from build123d import *

# Parameters (mm, degrees)
SKETCH1_W             = 100
SKETCH1_H             = 100
BOSS_EXTRUDE1_DEPTH   = 10
SKETCH2_W             = 50
SKETCH2_H             = 10
CUT_EXTRUDE1_DEPTH    = 113.249721603
SKETCH3_W             = 50
SKETCH3_H             = 10
CUT_EXTRUDE2_DEPTH    = 113.249721603
FILLET1_R             = 10
SKETCH5_R             = 30
BOSS_EXTRUDE2_DEPTH   = 2
SKETCH6_W             = 50
SKETCH6_H             = 20
BOSS_EXTRUDE3_DEPTH   = 50
SKETCH7_W             = 50
SKETCH7_H             = 35
BOSS_EXTRUDE6_DEPTH   = 20
CHAMFER1_SIZE         = 2
M8_TAPPED_HOLE1_D     = 6.8
M8_TAPPED_HOLE1_DEPTH = 20.207073895
M8_TAPPED_HOLE1_TIP   = 2.042926105


with BuildPart() as part:
    # Sketch1 → Boss-Extrude1 (new body)
    with BuildSketch(Plane(origin=(0, 0, 0), x_dir=(1, 0, 0), z_dir=(0, 1, 0))):
        Rectangle(SKETCH1_W, SKETCH1_H)
    extrude(amount=BOSS_EXTRUDE1_DEPTH)

    # Sketch2 → Cut-Extrude1 (cut, through all)
    with BuildSketch(Plane.XY.offset(50)):
        Rectangle(SKETCH2_W, SKETCH2_H)
    extrude(amount=-CUT_EXTRUDE1_DEPTH, mode=Mode.SUBTRACT)

    # Sketch3 → Cut-Extrude2 (cut, through all)
    with BuildSketch(Plane(origin=(50, 0, 0), x_dir=(0, 0, -1), z_dir=(1, 0, 0))):
        Rectangle(SKETCH3_W, SKETCH3_H)
    extrude(amount=-CUT_EXTRUDE2_DEPTH, mode=Mode.SUBTRACT)

    # Fillet1
    fillet1_edges = [part.edges().sort_by_distance(p)[0] for p in [
        (50, 5, 50),
        (-50, 5, 50),
        (-50, 5, -50),
        (50, 5, -50),
    ]]
    fillet(fillet1_edges, radius=FILLET1_R)

    # Sketch4 → Revolve1 (revolve)
    with BuildSketch(Plane.XY):
        Polygon((0, 10), (0, 30), (30, 30), (40, 10), align=None)
    revolve(axis=Axis((0, 10, 0), (0, 1, 0)))

    # Sketch5 → Boss-Extrude2 (add)
    with BuildSketch(Plane(origin=(0, 30, 0), x_dir=(1, 0, 0), z_dir=(0, 1, 0))):
        with Locations(Location((0, 0, 0), (0, 0, 180))):
            Circle(SKETCH5_R)
    extrude(amount=BOSS_EXTRUDE2_DEPTH)

    # Sketch6 → Boss-Extrude3 (add)
    with BuildSketch(Plane(origin=(0, 0, 0), x_dir=(0, 0, -1), z_dir=(1, 0, 0))):
        with Locations((0, 20)):
            Rectangle(SKETCH6_W, SKETCH6_H)
    extrude(amount=BOSS_EXTRUDE3_DEPTH)

    # Sketch7 → Boss-Extrude6 (add)
    with BuildSketch(Plane(origin=(50, 0, 0), x_dir=(0, 0, -1), z_dir=(1, 0, 0))):
        with Locations((0, 22.5)):
            Rectangle(SKETCH7_W, SKETCH7_H)
    extrude(amount=BOSS_EXTRUDE6_DEPTH)

    # Chamfer1
    chamfer1_edges = [part.edges().sort_by_distance(p)[0] for p in [
        (70, 5, 0),
        (50, 40, 0),
        (60, 5, -25),
        (50, 35, -25),
        (60, 40, -25),
        (70, 22.5, -25),
        (70, 40, 0),
        (60, 5, 25),
        (70, 22.5, 25),
        (60, 40, 25),
        (50, 35, 25),
    ]]
    chamfer(chamfer1_edges, length=CHAMFER1_SIZE)

    # M8 Tapped Hole1
    with Locations(Plane(origin=(0, 10, 0), x_dir=(1, 0, 0), z_dir=(0, 1, 0))):
        with Locations((40, 40), (40, -40), (-40, -40), (-40, 40)):
            Hole(M8_TAPPED_HOLE1_D / 2, depth=M8_TAPPED_HOLE1_DEPTH)
            with Locations((0, 0, -(M8_TAPPED_HOLE1_DEPTH + M8_TAPPED_HOLE1_TIP / 2))):  # 118° drill point
                Cone(0, M8_TAPPED_HOLE1_D / 2, M8_TAPPED_HOLE1_TIP, mode=Mode.SUBTRACT)


solid = part.part
Verification items for the finished model (mm, model axes). A direction names the side the tool comes from. Coordinates: 2 decimals unless noted, no trailing zeros. Order: outer loops, then holes, each group sorted by start corner. A loop starts at its lowest first (then second) coordinate and runs counter-clockwise, first axis right, second up.
Item 1: Section check D-D, the plane x = 55. Enter the section's corners in (y, z), then the cut area to 3 significant figures.
Filled in:
outline: (5, -23) - (7, -25) - (38, -25) - (40, -23) - (40, 23) - (38, 25) - (7, 25) - (5, 23) - close
area: 1,740 mm2
Item 2: Access from +Z, -Z, +X, -X, +Y, -Y to the whole of each face (thin tool, end or side, straight path). Record for faces 1 (the face through (38, 2, -25)), 2 (the face through (0, 32, 0)), 3 (the face through (-34, 10, -23)).
Filled in:
face 1: +X, -X, -Y
face 2: +Z, -Z, -X, +Y
face 3: +Y
Item 3: Section check C-C, the plane y = 18.5. Enter the section's corners in (x, z), then the cut area to 3 significant figures.
Filled in:
outline: (25.56, -25) - (68, -25) - (70, -23) - (70, 23) - (68, 25) - (25.56, 25) arc R35.75 ccw (long way) to start
area: 5,880 mm2
Item 4: Release check for a two-part mould opening along X. For faces 4 (the face through (48, 22, -25)), 5 (the face through (50, 5, 32)), 6 (the face through (-25, 2, -37)) record: +X half, -X half, draft (parallel to the pull), parting line (faces both ways), or undercut.
Filled in:
face 4: draft
face 5: +X half
face 6: undercut
Item 5: Section check A-A, the plane x = 0. Enter the section's corners in (y, z), then the cut area to 3 significant figures.
Filled in:
outline: (5, -50) - (10, -50) - (10, -40) - (30, -30) - (32, -30) - (32, 30) - (30, 30) - (10, 40) - (10, 50) - (5, 50) - close
area: 2,020 mm2
Item 6: Depth check by flat-ended pin: pin 1 (1 mm diameter, centred on x = 45, z = -37.5, fed in from +Y); pin 2 (2.5 mm diameter, centred on y = 2.5, z = -38.5, fed in from +X); pin 3 (18 mm diameter, centred on x = -6.5, z = 0, fed in from +Y); pin 4 (5 mm diameter, centred on x = 4, y = 36, fed in from +Z). Enter the tip coordinate at first touch or a pass-through.
Filled in:
pin 1: stops at y = 10
pin 2: stops at x = 50
pin 3: stops at y = 32
pin 4: passes through
Item 7: Section check B-B, the plane z = 0. Enter the section's corners in (x, y), then the cut area to 3 significant figures.
Filled in:
outline: (-50, 5) - (68, 5) - (70, 7) - (70, 38) - (68, 40) - (52, 40) - (50, 38) - (50, 30) - (30, 30) - (30, 32) - (-30, 32) - (-30, 30) - (-40, 10) - (-50, 10) - close
area: 3,010 mm2
Item 8: Material ranges on L1, parallel to X at y = 3.25, z = 40; L2, parallel to Z at x = -40, y = 5.75, recorded low to high.
Filled in:
L1: x = -50 to -43.4, -36.6 to -25, 25 to 36.6, 43.4 to 50
L2: z = -50 to -43.4, -36.6 to 36.6, 43.4 to 50
